Check sheet for the drawn part. Datum: minimum x, y, z corner. Units: mm. Round coordinates to 2 decimals unless told otherwise and drop trailing zeros. Write each loop counter-clockwise with the first axis right and the second up, starting at its lowest first coordinate (ties: lowest second). Pieces come first, ordered by that corner, then holes. Notation, with made-up numbers: (39, -7) - (46, -7) arc R27 cw to (46, 18) - close; hole circle Ø9 at (-23, -16). An arc over 180 degrees is marked (long way). Answer as a JSON object with one key per item and string values. Group by question number.
1) Section check D-D (y = 131.5). Enter the section's corners in (x, z), then the cut area to 3 significant figures.
2) Go/stop test with flat-tipped pins: pin 1 Ø2 at (x, z) = (133, 3.5) entering from +Y; pin 2 Ø15 at (y, z) = (447.5, 18.5) entering from -X; pin 3 Ø12 at (y, z) = (156.5, 4) entering from +X. Record where each tip stops, or that it passes through.
3) Section check C-C (x = 201). Enter the section's corners in (y, z).
4) Section check A-A (y = 369.5). Enter the section's corners in (x, z).
5) Section check B-B (z = 15). Enter the section's corners in (x, y).
6) Thickness scan on line 1 (Y direction, x = 114, z = 22.25); line 2 (Y direction, x = 413, z = 19.5) (1 decimal); line 3 (X direction, y = 384, z = 19.75). Record the ranges inside material, lowest first.
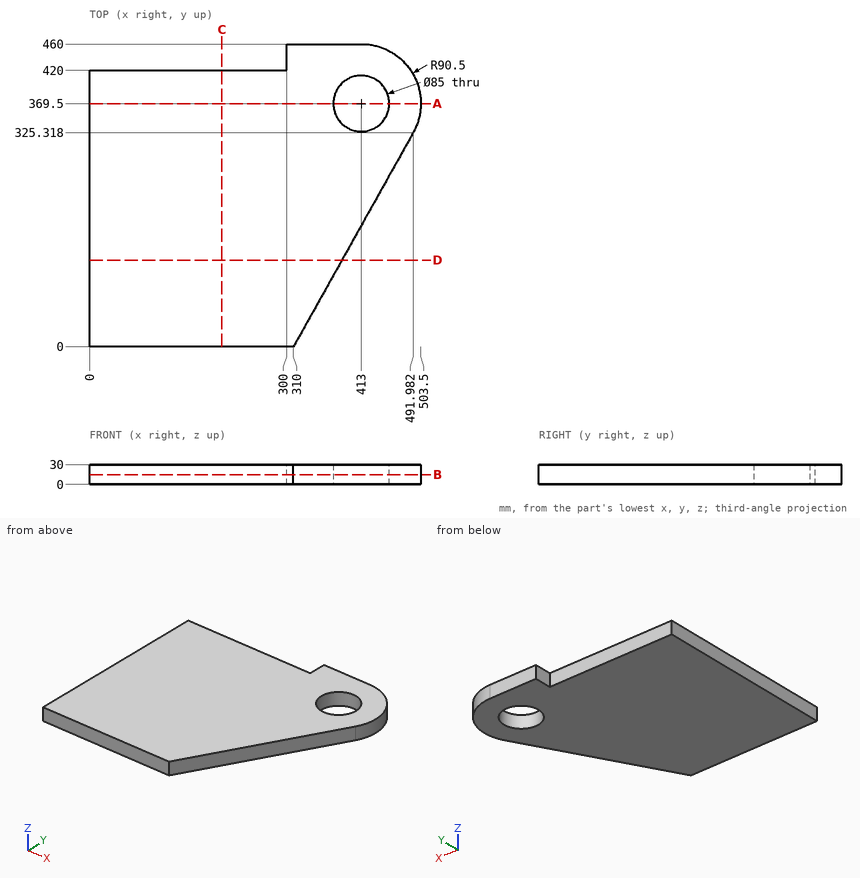
Returned:
{
 "1": {"outline": "(0, 0) - (383.56, 0) - (383.56, 30) - (0, 30) - close", "area": "11,500 mm2"},
 "2": {"pin 1": "y = 420", "pin 2": "x = 300", "pin 3": "x = 400.9"},
 "3": {"outline": "(0, 0) - (420, 0) - (420, 30) - (0, 30) - close"},
 "4": {"outline": "(0, 0) - (370.5, 0) - (370.5, 30) - (0, 30) - close; (455.5, 0) - (503.5, 0) - (503.5, 30) - (455.5, 30) - close"},
 "5": {"outline": "(0, 0) - (310, 0) - (491.98, 325.32) arc R90.5 ccw to (413, 460) - (300, 460) - (300, 420) - (0, 420) - close; hole circle Ø85 at (413, 369.5)"},
 "6": {"line 1": "0 to 420", "line 2": "184.1 to 327, 412 to 460", "line 3": "0 to 373.05, 452.95 to 502.33"}
}
